```python
from build123d import *

# Parameters (mm, degrees)
PLATE_AND_TUBE_PROFILE_SKETCH_R = 75
PLATE_AND_TUBE_BODY_DEPTH       = 250
MOUNTING_HOLES_4X_REACH         = 476.098
MOUNTING_HOLES_SKETCH_R         = 12.5


with BuildPart() as part:
    # Plate and Tube Profile Sketch → Plate and Tube Body (new body)
    with BuildSketch(Plane.XY):
        with BuildLine():
            Line((35.156791662, -16), (325, -16))
            Line((325, -16), (325, 16))
            Line((325, 16), (-325, 16))
            Line((-325, 16), (-325, -16))
            Line((-325, -16), (-35.156791662, -16))
            ThreePointArc((-35.156791662, -16), (0, -222), (35.156791662, -16))
        make_face()
        with Locations((0, -116)):
            Circle(PLATE_AND_TUBE_PROFILE_SKETCH_R, mode=Mode.SUBTRACT)
    extrude(amount=PLATE_AND_TUBE_BODY_DEPTH)

    # Mounting Holes Sketch → Mounting Holes 4x (cut, up to next)
    with BuildSketch(Plane(origin=(0, 16, 0), x_dir=(1, 0, 0), z_dir=(0, 1, 0)), mode=Mode.PRIVATE) as mounting_holes_4x_sk1:
        with Locations(Location((-250, -62.5, 0), (0, 0, 270))):
            Circle(MOUNTING_HOLES_SKETCH_R)
    mounting_holes_4x_tool1 = extrude(mounting_holes_4x_sk1.sketch, amount=-MOUNTING_HOLES_4X_REACH, mode=Mode.PRIVATE) & part.part
    # Mounting Holes Sketch → Mounting Holes 4x (cut, up to next)
    with BuildSketch(Plane(origin=(0, 16, 0), x_dir=(1, 0, 0), z_dir=(0, 1, 0)), mode=Mode.PRIVATE) as mounting_holes_4x_sk2:
        with Locations(Location((250, -62.5, 0), (0, 0, 270))):
            Circle(MOUNTING_HOLES_SKETCH_R)
    mounting_holes_4x_tool2 = extrude(mounting_holes_4x_sk2.sketch, amount=-MOUNTING_HOLES_4X_REACH, mode=Mode.PRIVATE) & part.part
    # Mounting Holes Sketch → Mounting Holes 4x (cut, up to next)
    with BuildSketch(Plane(origin=(0, 16, 0), x_dir=(1, 0, 0), z_dir=(0, 1, 0)), mode=Mode.PRIVATE) as mounting_holes_4x_sk3:
        with Locations(Location((-250, -187.5, 0), (0, 0, 270))):
            Circle(MOUNTING_HOLES_SKETCH_R)
    mounting_holes_4x_tool3 = extrude(mounting_holes_4x_sk3.sketch, amount=-MOUNTING_HOLES_4X_REACH, mode=Mode.PRIVATE) & part.part
    # Mounting Holes Sketch → Mounting Holes 4x (cut, up to next)
    with BuildSketch(Plane(origin=(0, 16, 0), x_dir=(1, 0, 0), z_dir=(0, 1, 0)), mode=Mode.PRIVATE) as mounting_holes_4x_sk4:
        with Locations(Location((250, -187.5, 0), (0, 0, 270))):
            Circle(MOUNTING_HOLES_SKETCH_R)
    mounting_holes_4x_tool4 = extrude(mounting_holes_4x_sk4.sketch, amount=-MOUNTING_HOLES_4X_REACH, mode=Mode.PRIVATE) & part.part
    add(mounting_holes_4x_tool1.solids().sort_by_distance((-250, 16, 62.5))[0], mode=Mode.SUBTRACT)
    add(mounting_holes_4x_tool2.solids().sort_by_distance((250, 16, 62.5))[0], mode=Mode.SUBTRACT)
    add(mounting_holes_4x_tool3.solids().sort_by_distance((-250, 16, 187.5))[0], mode=Mode.SUBTRACT)
    add(mounting_holes_4x_tool4.solids().sort_by_distance((250, 16, 187.5))[0], mode=Mode.SUBTRACT)


solid = part.part
```
Here's how the part is built. I have some questions about the finished solid (model axes, mm). A direction names the side the tool comes from. Round coordinates to 2 decimals unless told otherwise and drop trailing zeros. Order: outer loops, then holes, each group sorted by start corner. A loop starts at its lowest first (then second) coordinate and runs counter-clockwise, first axis right, second up. Notation, with made-up numbers: (78, -38) -> (127, -38) arc R24 cw to (127, -18) -> close; hole circle Ø1 at (46, -20). An arc over 180 degrees is marked (long way). Use a Markdown table: item, result. Add a question column.
(1) For faces 1 (the face through (-239.46, 0.22, 194.22)), 2 (the face through (-182, -16, 123)), which set-ups out of +Z, -Z, +X, -X, +Y, -Y let a thin tool reach every point of the face, with its end or its side?
(2) For pin 1 Ø20 at (x, z) = (250, 62.5) entering from -Y; pin 2 Ø3 at (x, z) = (-191.5, 209) entering from -Y; pin 3 Ø4 at (y, z) = (-81.5, 170) entering from +X; pin 4 Ø8 at (y, z) = (-141, 147) entering from +X, each with a flat end and sliding along its axis, tell me the tip position at first contact or that it passes through.
(3) I need wall thicknesses on line 1 along X through (y, z) = (-8, 187.5); line 2 along X through (y, z) = (-15, 191); line 3 along Y through (x, z) = (53.5, 188.5). Which ranges of each line are inside material? Lowest first, please.
(4) Suppose I cut it at B-B, the plane x = 0. Please give me the cut outline in (y, z), and give its area (3 significant figures).
(5) Suppose I cut it at A-A, the plane z = 62.5. Please give me the cut outline in (x, y).
(6) Suppose I cut it at C-C, the plane y = -116. Please give me the cut outline in (x, z), and give its area (3 significant figures).
(7) If we mould it in two halves opening along Z, with no side actions, what happens to faces 3 (the face through (325, 0, 123)), 4 (the face through (253.755, 0.224, 199.423)), 5 (the face through (262.394, 0.224, 60.873)), 6 (the face through (-1.5, -40.7, 250))? For each: released by +Z, released by -Z, zero draft, split by the parting line, or undercut.
(8) Suppose I cut it at D-D, the plane x = 250. Please give me the cut outline in (y, z), and give its area (3 significant figures).
Verdict:
| question | item | result |
|---|---|---|
| 1 | face 1 | +Y, -Y |
| 1 | face 2 | +Z, -Z, -X |
| 2 | pin 1 | through |
| 2 | pin 2 | y = -16 |
| 2 | pin 3 | x = 100.89 |
| 2 | pin 4 | x = 103.9 |
| 3 | line 1 | -325 to -262.5, -237.5 to 237.5, 262.5 to 325 |
| 3 | line 2 | -325 to -262, -238 to 238, 262 to 325 |
| 3 | line 3 | -207.51 to -168.56, -63.44 to -24.49, -16 to 16 |
| 4 | outline | (-222, 0) -> (-191, 0) -> (-191, 250) -> (-222, 250) -> close; (-41, 0) -> (16, 0) -> (16, 250) -> (-41, 250) -> close |
| 4 | area | 22,000 mm2 |
| 5 | outline | (-325, -16) -> (-262.5, -16) -> (-262.5, 16) -> (-325, 16) -> close; (-237.5, -16) -> (-35.16, -16) arc R106 ccw (long way) to (35.16, -16) -> (237.5, -16) -> (237.5, 16) -> (-237.5, 16) -> close; (262.5, -16) -> (325, -16) -> (325, 16) -> (262.5, 16) -> close; hole circle Ø150 at (0, -116) |
| 6 | outline | (-106, 0) -> (-75, 0) -> (-75, 250) -> (-106, 250) -> close; (75, 0) -> (106, 0) -> (106, 250) -> (75, 250) -> close |
| 6 | area | 15,500 mm2 |
| 7 | face 3 | zero draft |
| 7 | face 4 | undercut |
| 7 | face 5 | undercut |
| 7 | face 6 | released by +Z |
| 8 | outline | (-16, 0) -> (16, 0) -> (16, 50) -> (-16, 50) -> close; (-16, 75) -> (16, 75) -> (16, 175) -> (-16, 175) -> close; (-16, 200) -> (16, 200) -> (16, 250) -> (-16, 250) -> close |
| 8 | area | 6,400 mm2 |
